Design review of the part shown in the three views and the two pictorial views. Dimensions are in mm from the part's minimum x, y and z. Round coordinates to 2 decimals unless told otherwise and drop trailing zeros. Order: outer loops, then holes, each group sorted by start corner. A loop starts at its lowest first (then second) coordinate and runs counter-clockwise, first axis right, second up.
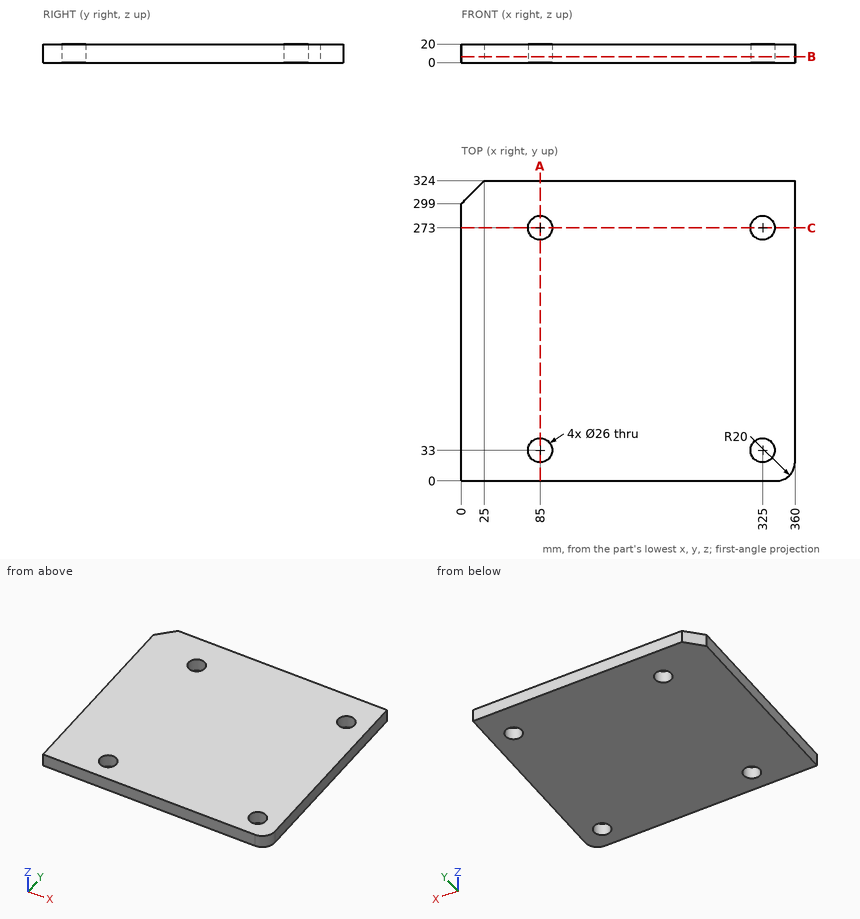
(1) To check wall thickness, follow probe 1 along Y at (x, z) = (325, 11); probe 2 along X at (y, z) = (37.5, 1.75); probe 3 along Y at (x, z) = (333.5, 11). State the ranges of each line that lie inside material, in increasing order.
Data:
probe 1: y = 0 to 20, 46 to 260, 286 to 324
probe 2: x = 0 to 72.8, 97.2 to 312.8, 337.2 to 360
probe 3: y = 0 to 23.16, 42.84 to 263.16, 282.84 to 324
(2) Insertion check: pin 1 (21 mm diameter, centred on x = 85, y = 273, fed in from -Z). The pin has a flat end and moves straight along its axis. Give the tip position at first contact, or say it passes through.
Data:
pin 1: passes through
(3) Consider section C-C (y = 273). Write out the cut boundary in (x, z), and give its area (3 significant figures).
Data:
outline: (0, 0) - (72, 0) - (72, 20) - (0, 20) - close; (98, 0) - (312, 0) - (312, 20) - (98, 20) - close; (338, 0) - (360, 0) - (360, 20) - (338, 20) - close
area: 6,160 mm2
(4) Consider section B-B (z = 6.5). Write out the cut boundary in (x, y).
Data:
outline: (0, 0) - (340, 0) arc R20 ccw to (360, 20) - (360, 324) - (25, 324) - (0, 299) - close; hole circle Ø26 at (85, 33); hole circle Ø26 at (85, 273); hole circle Ø26 at (325, 33); hole circle Ø26 at (325, 273)
(5) Consider section A-A (x = 85). Write out the cut boundary in (y, z), and give its area (3 significant figures).
Data:
outline: (0, 0) - (20, 0) - (20, 20) - (0, 20) - close; (46, 0) - (260, 0) - (260, 20) - (46, 20) - close; (286, 0) - (324, 0) - (324, 20) - (286, 20) - close
area: 5,440 mm2
